Work out the finished part from the listing and answer in its coordinate system (mm). A direction names the side the tool comes from. Give positions to 0.01 mm unless a question says otherwise; leave off trailing zeros. Order: outer loops, then holes, each group sorted by start corner. A loop starts at its lowest first (then second) coordinate and runs counter-clockwise, first axis right, second up. Notation, with made-up numbers: (78.25, -3) -> (84.25, -3) arc R23 cw to (84.25, 35) -> close; hole circle Ø2 at (81, -25). An arc over 180 degrees is marked (long way). Answer as CSV lines item,"result". Start each with the question number.
1. A cutting plane is placed at A-A (z = 25). Give the vertices of the cut face in (x, y), then the cut area to 3 significant figures.
2. Find the intervals of material crossed by L1, parallel to X at y = 4, z = 26; L2, parallel to Z at x = -24.5, y = 54, in increasing order.
3. A cutting plane is placed at B-B (z = 38.5). Give the vertices of the cut face in (x, y).
4. For faces 4 (the cylindrical face through (-47.05, 5.07, 27.7)), 5 (the cylindrical face through (-18, 24, 31)), 6 (the flat face through (-1, 35, 10)), determine the directions among +Z, -Z, +X, -X, +Y, -Y from which every point of the face is accessible in a straight line to the end or side of a thin tool.
5. For a pull along Y with two mould halves and no side action, classify faces 1 (the flat face through (0, 60, 5)), 2 (the flat face through (7, 19, 52)), 3 (the cylindrical face through (25.8, 32.7, 5.1)) as released by +Y, released by -Y, zero draft, split by the parting line, or undercut.
6. A cutting plane is placed at D-D (z = 8.5). Give the vertices of the cut face in (x, y).
7. Flat-ended cylindrical pins translate along their axes: pin 1 (14 mm diameter, centred on x = 30.53, y = 36.39, fed in from +Z); pin 2 (6 mm diameter, centred on y = 36.5, z = 8, fed in from -X); pin 3 (9 mm diameter, centred on x = -50, z = 25, fed in from +Y); pin 4 (5 mm diameter, centred on x = 50, z = 25, fed in from +Y). Find the tip coordinate at first contact, or state that the pin passes through.
8. A cutting plane is placed at C-C (x = 50). Give the vertices of the cut face in (y, z), then the cut area to 3 significant figures.
from build123d import *

# Parameters (mm, degrees)
BASE_FLANGE_DEPTH      = 10
BEARING_HOUSING_DEPTH  = 42
BORE_40_SKETCH_R       = 20
BORE_40_DEPTH          = 177
BACK_PLATE_DEPTH       = 10
BACK_PLATE_TRIM_DEPTH  = 10
HOLES_2X_8_SKETCH_R    = 4
HOLES_2X_8_DEPTH       = 56
HOLES_2X_12_SKETCH_R   = 6
HOLES_2X_12_DEPTH      = 56
HINGE_BOSS_18_SKETCH_R = 9
HINGE_BOSS_18_DEPTH    = 50
PIN_HOLE_7_SKETCH_R    = 3.5
PIN_HOLE_7_DEPTH       = 75


with BuildPart() as part:
    # Base Flange Sketch → Base Flange (new body)
    with BuildSketch(Plane.XY):
        with BuildLine():
            Line((-62.5, 0), (0, 0))
            Line((0, 0), (38.178366278, 0))
            Line((38.178366278, 0), (62.5, 0))
            ThreePointArc((62.5, 0), (50, 37.5), (17.5, 60))
            Line((17.5, 60), (0, 60))
            Line((0, 60), (-17.5, 60))
            ThreePointArc((-17.5, 60), (-50, 37.5), (-62.5, 0))
        make_face()
    extrude(amount=BASE_FLANGE_DEPTH)

    # Bearing Housing Sketch → Bearing Housing (add)
    with BuildSketch(Plane.XY.offset(10)):
        with BuildLine():
            Line((30, 0), (62.5, 0))
            ThreePointArc((62.5, 0), (62.298378138, 5.016181951), (61.694813396, 10))
            Line((61.694813396, 10), (28.284271247, 10))
            ThreePointArc((28.284271247, 10), (29.56795679, 5.073059362), (30, 0))
        make_face()
        with BuildLine():
            Line((-30, 0), (30, 0))
            ThreePointArc((30, 0), (29.56795679, 5.073059362), (28.284271247, 10))
            ThreePointArc((28.284271247, 10), (0, 30), (-28.284271247, 10))
            ThreePointArc((-28.284271247, 10), (-29.56795679, 5.073059362), (-30, 0))
        make_face()
        with BuildLine():
            Line((-62.5, 0), (-30, 0))
            ThreePointArc((-30, 0), (-29.56795679, 5.073059362), (-28.284271247, 10))
            Line((-28.284271247, 10), (-61.694813396, 10))
            ThreePointArc((-61.694813396, 10), (-62.298378138, 5.016181951), (-62.5, 0))
        make_face()
    extrude(amount=BEARING_HOUSING_DEPTH)

    # Bore Ø40 Sketch → Bore Ø40 (cut)
    with BuildSketch(Plane.XY.offset(52)):
        Circle(BORE_40_SKETCH_R)
    extrude(amount=-BORE_40_DEPTH, mode=Mode.SUBTRACT)

    # Back Plate Sketch → Back Plate (add)
    with BuildSketch(Plane(origin=(0, 10, 0), x_dir=(1, 0, 0), z_dir=(0, 1, 0))):
        Polygon((61.694813396, -52), (67.5, -52), (67.5, 0), (62.5, 0), (61.694813396, 0), align=None)
        Polygon((-67.5, -52), (-61.694813396, -52), (-61.694813396, 0.006233525), (-67.5, 0.096123111), align=None)
    extrude(amount=-BACK_PLATE_DEPTH)

    # Back Plate Trim Sketch → Back Plate Trim (cut)
    with BuildSketch(Plane(origin=(0, 10, 0), x_dir=(1, 0, 0), z_dir=(0, 1, 0))):
        Polygon((67.5, -30), (35, -52), (67.5, -52), align=None)
        Polygon((-67.5, -52), (-67.5, -29.903876889), (-35, -52), align=None)
    extrude(amount=-BACK_PLATE_TRIM_DEPTH, mode=Mode.SUBTRACT)

    # Holes 2xØ8 Sketch → Holes 2xØ8 (cut)
    with BuildSketch(Plane(origin=(0, 10, 0), x_dir=(1, 0, 0), z_dir=(0, 1, 0))):
        with Locations(Location((50, -25, 0), (0, 0, 270))):
            Circle(HOLES_2X_8_SKETCH_R)
        with Locations(Location((-50, -25, 0), (0, 0, 180))):
            Circle(HOLES_2X_8_SKETCH_R)
    extrude(amount=-HOLES_2X_8_DEPTH, mode=Mode.SUBTRACT)

    # Holes 2xØ12 Sketch → Holes 2xØ12 (cut)
    with BuildSketch(Plane.XY.offset(10)):
        with Locations((30.53241146, 36.387111048)):
            Circle(HOLES_2X_12_SKETCH_R)
        with Locations((-30.53241146, 36.387111048)):
            Circle(HOLES_2X_12_SKETCH_R)
    extrude(amount=-HOLES_2X_12_DEPTH, mode=Mode.SUBTRACT)

    # Hinge Boss Ø18 Sketch → Hinge Boss Ø18 (add)
    with BuildSketch(Plane.XY.offset(52)):
        with Locations((7.764571353, 28.977774789)):
            Circle(HINGE_BOSS_18_SKETCH_R)
    extrude(amount=-HINGE_BOSS_18_DEPTH)

    # Pin Hole Ø7 Sketch → Pin Hole Ø7 (cut)
    with BuildSketch(Plane.XY.offset(52)):
        with Locations((7.764571353, 28.977774789)):
            Circle(PIN_HOLE_7_SKETCH_R)
    extrude(amount=-PIN_HOLE_7_DEPTH, mode=Mode.SUBTRACT)


solid = part.part
Answer sheet:
1,outline,"(-67.5, 0) -> (-54, 0) -> (-54, 10) -> (-67.5, 10) -> close; (-46, 0) -> (-20, 0) arc R20 cw to (20, 0) -> (46, 0) -> (46, 10) -> (28.28, 10) arc R30 ccw to (16.01, 25.37) arc R9 ccw (long way) to (-1.18, 29.98) arc R30 ccw to (-28.28, 10) -> (-46, 10) -> close; (54, 0) -> (67.5, 0) -> (67.5, 10) -> (54, 10) -> close; hole circle Ø7 at (7.76, 28.98)"
1,area,"1,480 mm^2"
2,L1,"x = -67.5 to -53.87, -46.13 to -19.6, 19.6 to 46.13, 53.87 to 67.5"
2,L2,"z = 0 to 10"
3,outline,"(-54.86, 0) -> (-20, 0) arc R20 cw to (20, 0) -> (54.94, 0) -> (54.94, 10) -> (28.28, 10) arc R30 ccw to (16.01, 25.37) arc R9 ccw (long way) to (-1.18, 29.98) arc R30 ccw to (-28.28, 10) -> (-54.86, 10) -> close; hole circle Ø7 at (7.76, 28.98)"
4,face 4,"+Y, -Y"
4,face 5,"+Z, -X, +Y"
4,face 6,"+Z, +Y"
5,face 1,"released by +Y"
5,face 2,"zero draft"
5,face 3,"undercut"
6,outline,"(-67.5, 0) -> (-20, 0) arc R20 cw to (20, 0) -> (67.5, 0) -> (67.5, 10) -> (61.69, 10) arc R62.5 ccw to (17.5, 60) -> (-17.5, 60) arc R62.5 ccw to (-61.69, 10) -> (-67.5, 10) -> close; hole circle Ø12 at (-30.53, 36.39); hole circle Ø7 at (7.76, 28.98); hole circle Ø12 at (30.53, 36.39)"
7,pin 1,"stops at z = 10"
7,pin 2,"stops at x = -52.76"
7,pin 3,"stops at y = 10"
7,pin 4,"passes through"
8,outline,"(0, 0) -> (37.5, 0) -> (37.5, 10) -> (10, 10) -> (10, 21) -> (0, 21) -> close; (0, 29) -> (10, 29) -> (10, 41.85) -> (0, 41.85) -> close"
8,area,"613 mm^2"
